Input: part model. Units: mm. Frame: model coordinates. Round coordinates to 2 decimals unless told otherwise and drop trailing zeros. Write each loop counter-clockwise with the first axis right and the second up, starting at its lowest first coordinate (ties: lowest second). Pieces come first, ordered by that corner, then holes. Notation, with made-up numbers: M 48,71.5 L 106,71.5 A28 cw 106,91.5 Z; hole C 4.5,-0.5 d9. An arc over 180 degrees is marked long. Answer as CSV lines item,"result". Start each with the question number.
```python
from build123d import *

# Parameters (mm, degrees)
SKETCH1_W                                            = 73.5
SKETCH1_H                                            = 50
BOSS_EXTRUDE1_DEPTH                                  = 13.5
CBORE_FOR_M4_HEXAGON_SOCKET_HEAD_CAP_SCR_D           = 4.5
CBORE_FOR_M4_HEXAGON_SOCKET_HEAD_CAP_SCR_CBORE_D     = 8
CBORE_FOR_M4_HEXAGON_SOCKET_HEAD_CAP_SCR_CBORE_DEPTH = 4.6
F_4_0MM_DOWEL_HOLE1_D                                = 4
F_4_0MM_DOWEL_HOLE1_DEPTH                            = 6
F_4_0MM_DOWEL_HOLE1_TIP                              = 1.201721238
M4_TAPPED_HOLE1_D                                    = 3.3
M4_TAPPED_HOLE1_DEPTH                                = 10.1
M4_TAPPED_HOLE1_TIP                                  = 0.991420021
CHAMFER1_SIZE                                        = 3


with BuildPart() as part:
    # Sketch1 → Boss-Extrude1 (new body)
    with BuildSketch(Plane(origin=(0, 0, 0), x_dir=(0, 0, -1), z_dir=(1, 0, 0))):
        Rectangle(SKETCH1_W, SKETCH1_H)
    extrude(amount=BOSS_EXTRUDE1_DEPTH)

    # CBORE for M4 Hexagon socket head cap screws1 (through all)
    with Locations(Plane.ZY):
        with Locations((30, -20), (30, 20), (-30, 20), (-30, -20)):
            CounterBoreHole(CBORE_FOR_M4_HEXAGON_SOCKET_HEAD_CAP_SCR_D / 2, CBORE_FOR_M4_HEXAGON_SOCKET_HEAD_CAP_SCR_CBORE_D / 2, CBORE_FOR_M4_HEXAGON_SOCKET_HEAD_CAP_SCR_CBORE_DEPTH)

    # Ø4.0mm Dowel Hole1
    with Locations(Plane(origin=(13.5, 0, 0), x_dir=(0, 0, -1), z_dir=(1, 0, 0))):
        with Locations((30, 0), (-30, 0)):
            Hole(F_4_0MM_DOWEL_HOLE1_D / 2, depth=F_4_0MM_DOWEL_HOLE1_DEPTH)
            with Locations((0, 0, -(F_4_0MM_DOWEL_HOLE1_DEPTH + F_4_0MM_DOWEL_HOLE1_TIP / 2))):  # 118° drill point
                Cone(0, F_4_0MM_DOWEL_HOLE1_D / 2, F_4_0MM_DOWEL_HOLE1_TIP, mode=Mode.SUBTRACT)

    # M4 Tapped Hole1
    with Locations(Plane.ZY):
        with Locations((28.25, -11.25), (-30.75, -11.25)):
            Hole(M4_TAPPED_HOLE1_D / 2, depth=M4_TAPPED_HOLE1_DEPTH)
            with Locations((0, 0, -(M4_TAPPED_HOLE1_DEPTH + M4_TAPPED_HOLE1_TIP / 2))):  # 118° drill point
                Cone(0, M4_TAPPED_HOLE1_D / 2, M4_TAPPED_HOLE1_TIP, mode=Mode.SUBTRACT)

    # Chamfer1
    chamfer1_edges = [part.edges().sort_by_distance(p)[0] for p in [
        (6.75, -25, -36.75),
        (6.75, -25, 36.75),
        (6.75, 25, 36.75),
        (6.75, 25, -36.75),
    ]]
    chamfer(chamfer1_edges, length=CHAMFER1_SIZE)


solid = part.part
```
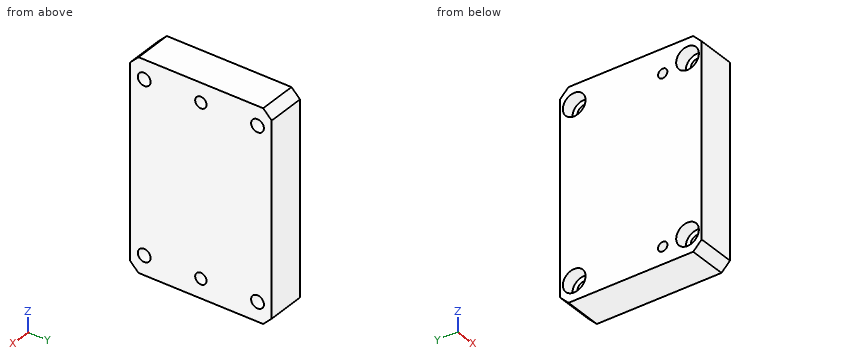
Item 1: Cut plane A-A, the plane x = 5.5. Return loops of the section in (y, z).
Item 2: Cut plane C-C, the plane z = -27. Return loops of the section in (x, y), plus the area to 3 significant figures.
Item 3: Cut plane B-B, the plane y = -20. Return loops of the section in (x, z).
Item 4: Cut plane D-D, the plane y = 21. Return loops of the section in (x, z), plus the area to 3 significant figures.
Item 5: Pin query (flat end, axial travel): pin 1 Ø5 at (y, z) = (20, 30) entering from -X; pin 2 Ø6.5 at (y, z) = (0, -30) entering from +X; pin 3 Ø2.5 at (y, z) = (-20.5, -29.5) entering from -X. Return the tip coordinate at first contact, or that it passes through.
Item 6: Line query: line 1 (Z direction, x = 4.5, y = -11.25); line 2 (Y direction, x = 5, z = 29); line 3 (Z direction, x = 11.5, y = -20.5). Output: solid intervals per line, ascending. Write a range as [from, to].
Results list:
1,outline,"M -25,-33.75 L -22,-36.75 L 22,-36.75 L 25,-33.75 L 25,33.75 L 22,36.75 L -22,36.75 L -25,33.75 Z; hole C -20,-30 d4.5; hole C -20,30 d4.5; hole C -11.25,-30.75 d3.3; hole C -11.25,28.25 d3.3; hole C 20,-30 d4.5; hole C 20,30 d4.5"
2,outline,"M 0,-25 L 13.5,-25 L 13.5,25 L 0,25 L 0,22.65 L 4.6,22.65 L 4.6,17.35 L 0,17.35 L 0,-17.35 L 4.6,-17.35 L 4.6,-22.65 L 0,-22.65 Z"
2,area,"626 mm²"
3,outline,"M 0,-36.75 L 13.5,-36.75 L 13.5,-32.25 L 4.6,-32.25 L 4.6,-34 L 0,-34 Z; M 0,-26 L 4.6,-26 L 4.6,-27.75 L 13.5,-27.75 L 13.5,27.75 L 4.6,27.75 L 4.6,26 L 0,26 Z; M 0,34 L 4.6,34 L 4.6,32.25 L 13.5,32.25 L 13.5,36.75 L 0,36.75 Z"
4,outline,"M 0,-36.75 L 13.5,-36.75 L 13.5,-32.02 L 4.6,-32.02 L 4.6,-33.87 L 0,-33.87 Z; M 0,-26.13 L 4.6,-26.13 L 4.6,-27.98 L 13.5,-27.98 L 13.5,27.98 L 4.6,27.98 L 4.6,26.13 L 0,26.13 Z; M 0,33.87 L 4.6,33.87 L 4.6,32.02 L 13.5,32.02 L 13.5,36.75 L 0,36.75 Z"
4,area,"849 mm²"
5,pin 1,"x = 4.6"
5,pin 2,"x = 13.5"
5,pin 3,"through"
6,line 1,"[-36.75, -32.4], [-29.1, 26.6], [29.9, 36.75]"
6,line 2,"[-25, -22.02], [-17.98, -12.72], [-9.78, 17.98], [22.02, 25]"
6,line 3,"[-36.75, -32.19], [-27.81, 27.81], [32.19, 36.75]"
